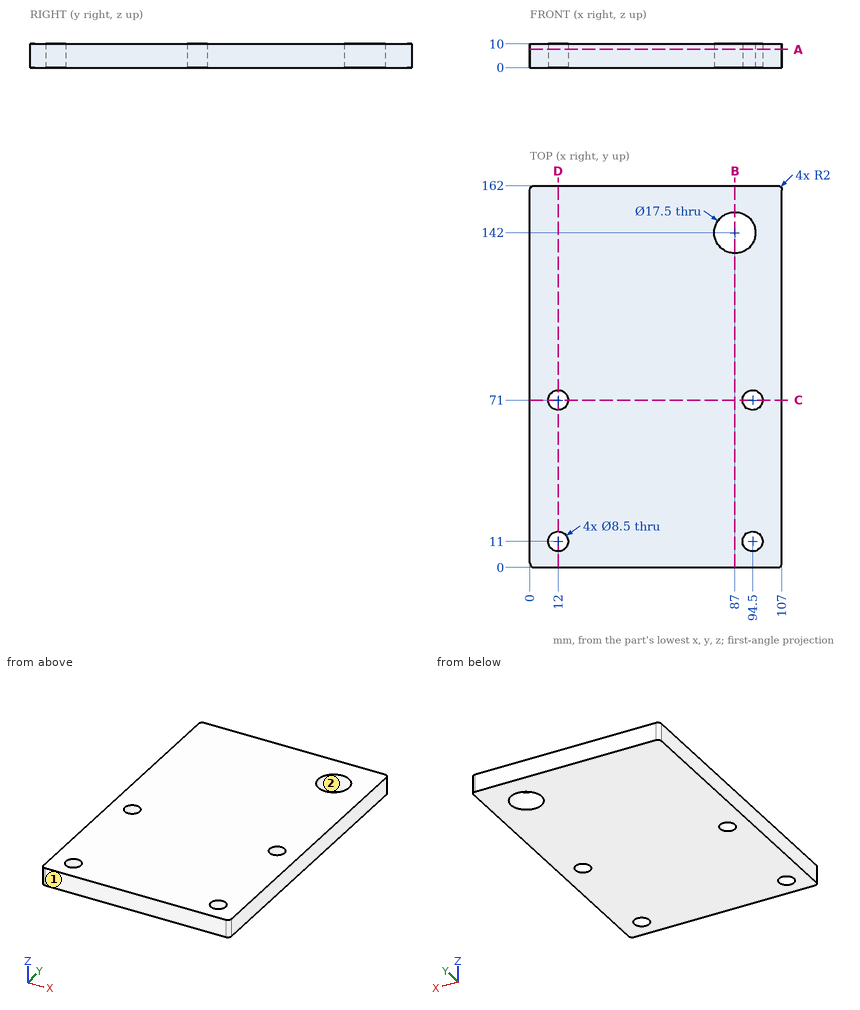
Design review of the part shown in the three views and the two pictorial views. Dimensions are in mm from the part's minimum x, y and z. Give positions to 0.01 mm unless a question says otherwise; leave off trailing zeros. Write each loop counter-clockwise with the first axis right and the second up, starting at its lowest first coordinate (ties: lowest second). Pieces come first, ordered by that corner, then holes. Notation, with made-up numbers: (55, 3.5) - (109, 3.5) arc R11 cw to (109, 20.5) - close; hole circle Ø2 at (19.25, 88). An arc over 180 degrees is marked (long way). Return JSON: item names as keys, results as strings. Group by question number.
(1) We need section D-D, the plane x = 12. Give the boundary of the cut face in (y, z), then the cut area to 3 significant figures.
(2) Mouldability with a two-part tool opening along X and no side actions: class the marked faces 1 and 2 as +X half, -X half, draft (parallel to the pull), parting line (faces both ways), or undercut.
(3) Insertion check: pin 1 (13.5 mm diameter, centred on x = 94.5, y = 71, fed in from +Z). The pin has a flat end and moves straight along its axis. Give the tip position at first contact, or say it passes through.
(4) We need section B-B, the plane x = 87. Give the boundary of the cut face in (y, z).
(5) To check wall thickness, follow probe 1 along Y at (x, z) = (12, 4); probe 2 along Y at (x, z) = (94.5, 3.75); probe 3 along X at (y, z) = (73, 5). State the ranges of each line that lie inside material, in increasing order.
(6) We need section C-C, the plane y = 71. Give the boundary of the cut face in (x, z), then the cut area to 3 significant figures.
(7) We need section A-A, the plane z = 7.75. Give the boundary of the cut face in (x, y).
Reported:
{
 "1": {"outline": "(0, 0) - (6.75, 0) - (6.75, 10) - (0, 10) - close; (15.25, 0) - (66.75, 0) - (66.75, 10) - (15.25, 10) - close; (75.25, 0) - (162, 0) - (162, 10) - (75.25, 10) - close", "area": "1,450 mm2"},
 "2": {"face 1": "draft", "face 2": "undercut"},
 "3": {"pin 1": "stops at z = 10"},
 "4": {"outline": "(0, 0) - (133.25, 0) - (133.25, 10) - (0, 10) - close; (150.75, 0) - (162, 0) - (162, 10) - (150.75, 10) - close"},
 "5": {"probe 1": "y = 0 to 6.75, 15.25 to 66.75, 75.25 to 162", "probe 2": "y = 0 to 6.75, 15.25 to 66.75, 75.25 to 137.49, 146.51 to 162", "probe 3": "x = 0 to 8.25, 15.75 to 90.75, 98.25 to 107"},
 "6": {"outline": "(0, 0) - (7.75, 0) - (7.75, 10) - (0, 10) - close; (16.25, 0) - (90.25, 0) - (90.25, 10) - (16.25, 10) - close; (98.75, 0) - (107, 0) - (107, 10) - (98.75, 10) - close", "area": "900 mm2"},
 "7": {"outline": "(0, 2) arc R2 ccw to (2, 0) - (105, 0) arc R2 ccw to (107, 2) - (107, 160) arc R2 ccw to (105, 162) - (2, 162) arc R2 ccw to (0, 160) - close; hole circle Ø8.5 at (12, 11); hole circle Ø8.5 at (12, 71); hole circle Ø17.5 at (87, 142); hole circle Ø8.5 at (94.5, 11); hole circle Ø8.5 at (94.5, 71)"}
}
